Build history of the part. All positions in model axes, mm. Face numbers are marked on the shaded views. Round coordinates to 2 decimals unless told otherwise and drop trailing zeros. Write each loop counter-clockwise with the first axis right and the second up, starting at its lowest first coordinate (ties: lowest second). Pieces come first, ordered by that corner, then holes. Notation, with made-up numbers: M -16,34.25 L -1,34.25 A6 ccw -1,42.25 Z; hole C 89,28.25 d10. An arc over 180 degrees is marked long. Write item = value, one per line. Start each with the question number.
Q1. Band-saw the part on C-C on y = 8. Write the cut outline in (x, z).
Q2. Band-saw the part on B-B on z = 0. Write the cut outline in (x, y), plus the area to 4 significant figures.
Q3. Pull direction X, two halves, no side cores. Call the marked faces 1, 2 and 3: released by +X, released by -X, zero draft, split by the parting line, or undercut.
Q4. Probe L1, parallel to Z at x = 0, y = 13.5; L2, parallel to X at y = 13, z = 0; L3, parallel to X at y = 5, z = 1.25. List the from-to ranges inside material, lowest first.
Q5. Band-saw the part on A-A on x = 0. Write the cut outline in (y, z), plus the area to 4 significant figures.
```python
from build123d import *

# Parameters (mm, degrees)
SKETCH1_W           = 25
SKETCH1_H           = 12
BOSS_EXTRUDE1_DEPTH = 18
SKETCH2_R           = 3
CUT_EXTRUDE1_DEPTH  = 23.721135535
CHAMFER1_SIZE       = 0.5


with BuildPart() as part:
    # Sketch1 → Boss-Extrude1 (new body)
    with BuildSketch(Plane(origin=(0, 0, 0), x_dir=(1, 0, 0), z_dir=(0, 1, 0))):
        Rectangle(SKETCH1_W, SKETCH1_H)
    extrude(amount=BOSS_EXTRUDE1_DEPTH)

    # Sketch2 → Cut-Extrude1 (cut, through all)
    with BuildSketch(Plane(origin=(0, 0, 0), x_dir=(1, 0, 0), z_dir=(0, 1, 0))):
        with Locations(Location((0, 0, 0), (0, 0, 270))):
            Circle(SKETCH2_R)
    extrude(amount=CUT_EXTRUDE1_DEPTH, mode=Mode.SUBTRACT)

    # Chamfer1
    chamfer1_edges = [part.edges().sort_by_distance(p)[0] for p in [
        (0, 0, -3),
        (0, 18, -3),
    ]]
    chamfer(chamfer1_edges, length=CHAMFER1_SIZE)


solid = part.part
```
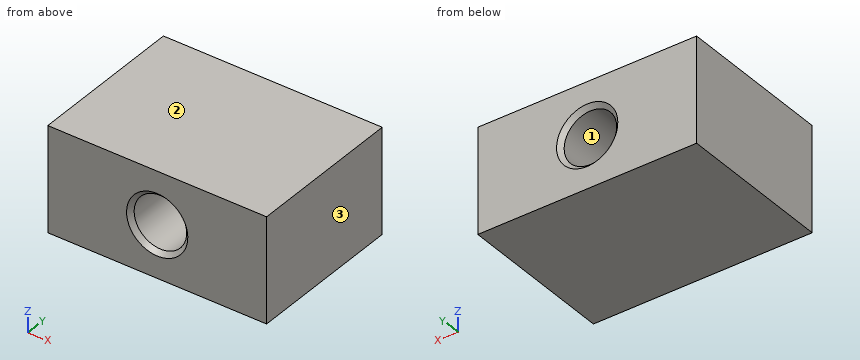
Conclusion:
q1.outline = M -12.5,-6 L 12.5,-6 L 12.5,6 L -12.5,6 Z; hole C 0,0 d6
q2.outline = M -12.5,0 L -3.5,0 L -3,0.5 L -3,17.5 L -3.5,18 L -12.5,18 Z; M 3,0.5 L 3.5,0 L 12.5,0 L 12.5,18 L 3.5,18 L 3,17.5 Z
q2.area = 341.5 mm^2
q3.face_1 = undercut
q3.face_2 = zero draft
q3.face_3 = released by +X
q4.L1 = -6 to -3, 3 to 6
q4.L2 = -12.5 to -3, 3 to 12.5
q4.L3 = -12.5 to -2.73, 2.73 to 12.5
q5.outline = M 0,-6 L 18,-6 L 18,-3.5 L 17.5,-3 L 0.5,-3 L 0,-3.5 Z; M 0,3.5 L 0.5,3 L 17.5,3 L 18,3.5 L 18,6 L 0,6 Z
q5.area = 107.5 mm^2
